Read the model definition and answer for the solid it produces. Units are mm, in the model's axes. Face numbers are marked on the shaded views. A direction names the side the tool comes from. Round coordinates to 2 decimals unless told otherwise and drop trailing zeros. Loops run counter-clockwise (first coordinate to the right, second up) from the corner with the lowest first, then second, coordinate; pieces in that order, holes last. Notation, with made-up numbers: (-2.75, 42.5) -> (51.25, 42.5) arc R23 ccw to (51.25, 62.5) -> close; hole circle Ø5 at (-17, 9). An arc over 180 degrees is marked (long way). Put each result on its own line as item: value.
from build123d import *

# Parameters (mm, degrees)
SKETCH_3_R               = 3.67
REVOLVE_2_ANGLE          = 90
EXTRUDE_1_DEPTH          = 5.8
CUT_EXTRUDE_1_DEPTH      = 14
CUT_EXTRUDE_1_DEPTH_BACK = 14
SKETCH_5_R               = 3


with BuildPart() as part:
    # 草图1 → 旋转1 (revolve)
    with BuildSketch(Plane.XY, mode=Mode.PRIVATE) as revolve_1_sk:
        Polygon((0, 0), (-2.01, 0), (-2.5, 0.49), (-2.5, 2.5), (-3.15, 2.5), (-3.15, 10.705), (0, 10.705), align=None)
    revolve(revolve_1_sk.sketch.rotate(Axis((0, 10.705, 0), (0, -1, 0)), 180), axis=Axis((0, 10.705, 0), (0, -1, 0)))

    # 草图3 → 旋转2 (revolve)
    with BuildSketch(Plane(origin=(0, 10.705, 0), x_dir=(1, 0, 0), z_dir=(0, 1, 0))):
        Circle(SKETCH_3_R)
    revolve(axis=Axis((3.68, 10.705, 3.795), (1, 0, 0)), revolution_arc=REVOLVE_2_ANGLE)

    # 草图4 → 凸台-拉伸1 (add)
    with BuildSketch(Plane(origin=(0, 3.25, 0), x_dir=(1, 0, 0), z_dir=(0, 1, 0))):
        Polygon((-3.5, 2.020725942), (-3.5, -2.020725942), (0, -4.041451884), (3.5, -2.020725942), (3.5, 2.020725942), (0, 4.041451884), align=None)
    extrude(amount=EXTRUDE_1_DEPTH)

    # 草图2 → 旋转3 (revolve)
    with BuildSketch(Plane(origin=(0, 14.5, 0), x_dir=(1, 0, 0), z_dir=(0, 1, 0)), mode=Mode.PRIVATE) as revolve_3_sk:
        Polygon((0, -16), (-5.75, -16), (-5.75, -14.5), (-4.5, -14.5), (-4.5, -14), (-5.75, -14), (-5.75, -4.554654828), (-3.68, -4), (-3.68, -3.565), (0, -3.565), align=None)
    revolve(revolve_3_sk.sketch.rotate(Axis((0, 14.5, 3.565), (0, 0, 1)), 180), axis=Axis((0, 14.5, 3.565), (0, 0, 1)))

    # 草图5 → 切除-拉伸1 (cut, two sides: drawn at the far end of the back side and taken through both)
    with BuildSketch(Plane.XY.offset(16).offset(-CUT_EXTRUDE_1_DEPTH_BACK)):
        with Locations(Location((0, 14.5, 0), (0, 0, 180))):
            Circle(SKETCH_5_R)
    extrude(amount=CUT_EXTRUDE_1_DEPTH + CUT_EXTRUDE_1_DEPTH_BACK, mode=Mode.SUBTRACT)


solid = part.part
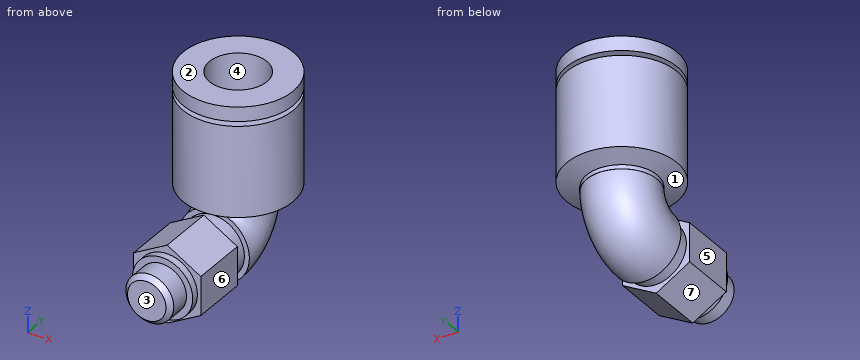
Item 1: Flat-ended cylindrical pins translate along their axes: pin 1 Ø4.5 at (y, z) = (6.5, 0.5) entering from +X; pin 2 Ø2 at (x, z) = (1.5, -1) entering from +Y; pin 3 Ø4 at (x, z) = (1, 6) entering from -Y. Find the tip coordinate at first contact, or state that the pin passes through.
Derived:
pin 1: stops at x = 3.5
pin 2: stops at y = 16.89
pin 3: stops at y = 8.75
Item 2: The part is cut by section A-A (y = 4). Determine the outline of the cut face in (x, z).
Derived:
outline: (-3.5, -2.02) -> (0, -4.04) -> (3.5, -2.02) -> (3.5, 2.02) -> (0, 4.04) -> (-3.5, 2.02) -> close
Item 3: Which of the six approach directions +Z, -Z, +X, -X, +Y, -Y give full straight-line access (tool end or side, diameter ignored) to the marked faces 4, 5, 6 and 7?
Derived:
face 4: +Z
face 5: +Z, -Z, -X, -Y
face 6: +Z, -Z, +X, -Y
face 7: -Z, -X, -Y
Item 4: The part is cut by section C-C (y = 1.5). Determine the outline of the cut face in (x, z).
Derived:
outline: circle Ø5 at (0, 0)
Item 5: For a pull along Z with two mould halves and no side action, classify the marked faces 1, 2 and 3 as pulls with the +Z half, pulls with the -Z half, needs draft (parallel to the pull), parting line crosses it, or undercut.
Derived:
face 1: undercut
face 2: pulls with the +Z half
face 3: needs draft
Item 6: Find the intervals of material crossed by line 1 along Y through (x, z) = (0, 12.75); line 2 along Z through (x, y) = (4.75, 13); line 3 along X through (y, z) = (16.5, 8.5), in increasing order.
Derived:
line 1: y = 8.75 to 11.5, 17.5 to 20.25
line 2: z = 4.35 to 14, 14.5 to 16
line 3: x = -5.39 to -2.24, 2.24 to 5.39
Item 7: The part is cut by section B-B (z = 11.25). Determine the outline of the cut face in (x, y).
Derived:
outline: circle Ø11.5 at (0, 14.5); hole circle Ø6 at (0, 14.5)
